Study the drawing (mm; zero at the part's minimum x, y, z) and answer. A direction names the side the tool comes from. Round coordinates to 2 decimals unless told otherwise and drop trailing zeros. Order: outer loops, then holes, each group sorted by start corner. A loop starts at its lowest first (then second) coordinate and runs counter-clockwise, first axis right, second up. Notation, with made-up numbers: (56, 26.5) - (78, 26.5) arc R31 ccw to (78, 56.5) - close; hole circle Ø6 at (-13.5, 76.25). An arc over 180 degrees is marked (long way). Put each result on its own line as item: value.
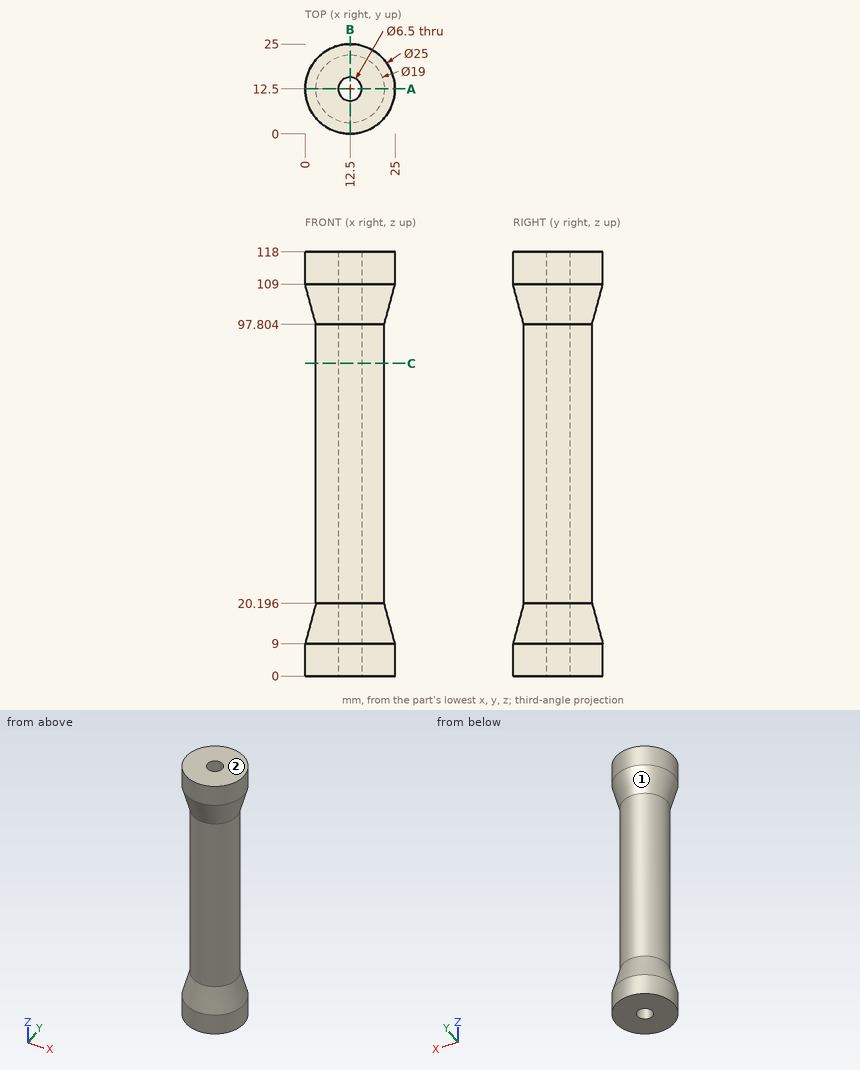
1) A cutting plane is placed at C-C on z = 87. Write down the section's boundary in (x, y).
Findings below:
outline: circle Ø19 at (12.5, 12.5); hole circle Ø6.5 at (12.5, 12.5)
2) A cutting plane is placed at A-A on y = 12.5. Write down the section's boundary in (x, z), then the cut area to 3 significant figures.
Findings below:
outline: (0, 0) - (9.25, 0) - (9.25, 118) - (0, 118) - (0, 109) - (3, 97.8) - (3, 20.2) - (0, 9) - close; (15.75, 0) - (25, 0) - (25, 9) - (22, 20.2) - (22, 97.8) - (25, 109) - (25, 118) - (15.75, 118) - close
area: 1,650 mm2
3) Given pin 1 Ø1.5 at (x, z) = (5, 60) entering from +Y (1 decimal); pin 2 Ø3 at (y, z) = (8.5, 83) entering from +X (3 decimals); pin 3 Ø1.5 at (y, z) = (17, 51) entering from -X, each flat-ended and moving along its own axis, determine where each tip first touches the part or whether it passes through.
Findings below:
pin 1: stops at y = 19.2
pin 2: stops at x = 21.665
pin 3: stops at x = 3.77
4) For the marked faces 1 and 2, determine the directions among +Z, -Z, +X, -X, +Y, -Y from which every point of the face is accessible in a straight line to the end or side of a thin tool.
Findings below:
face 1: none
face 2: +Z, +X, -X, +Y, -Y
5) Straight lines are drawn through the part: L1, parallel to Y at x = 12.5, z = 74.5; L2, parallel to Y at x = 15.25, z = 11 (1 decimal); L3, parallel to X at y = 14.75, z = 17 (1 decimal). For each, find the intervals that lie inside material, in ascending order. Write a range as from..to.
Findings below:
L1: y = 3..9.25, 15.75..22
L2: y = 0.9..10.8, 14.2..24.1
L3: x = 2.4..10.2, 14.8..22.6
